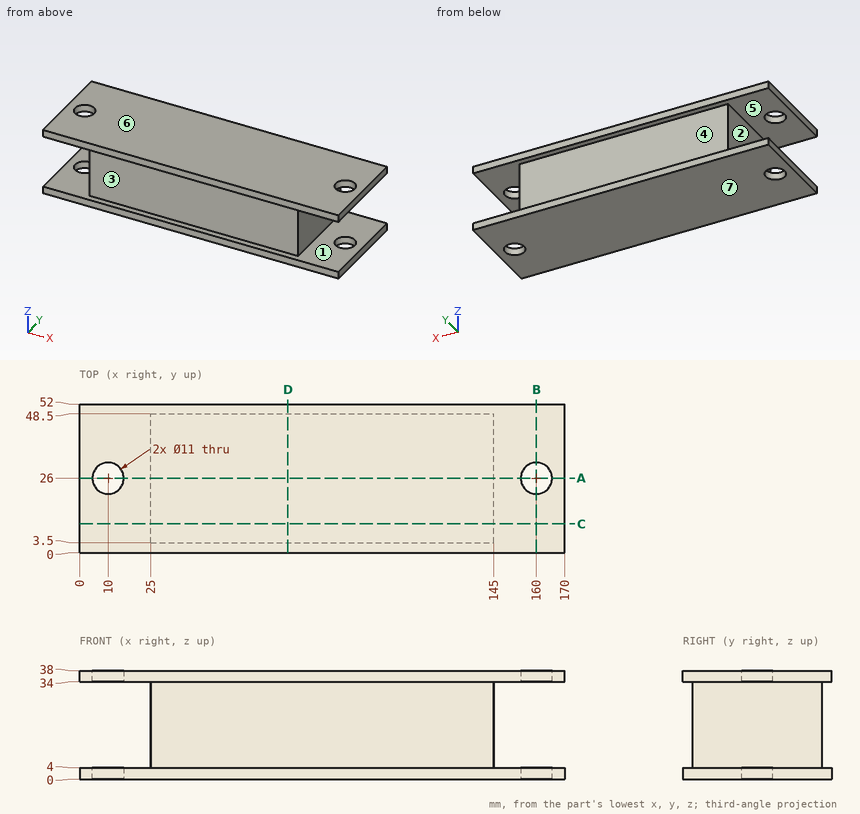
The drawing under review shows one solid part. Ordinate dimensions are in mm from its lowest x, y, z. A direction names the side the tool comes from. Coordinates: 2 decimals unless noted, no trailing zeros. Order: outer loops, then holes, each group sorted by start corner. A loop starts at its lowest first (then second) coordinate and runs counter-clockwise, first axis right, second up. Notation, with made-up numbers: (0.25, 74) -> (27.25, 74) arc R29 ccw to (27.25, 113) -> close; hole circle Ø1 at (5.5, 70.25). An arc over 180 degrees is marked (long way). Return JSON: item names as keys, results as strings.
1. For pin 1 Ø12 at (x, z) = (28, 23) entering from +Y; pin 2 Ø12 at (x, z) = (19, 33) entering from -Y; pin 3 Ø6 at (y, z) = (20, 25.5) entering from +X; pin 4 Ø8 at (x, z) = (133.5, 14.5) entering from -Y, all flat-tipped, find the tip position at first contact; note any pin that passes through.
Answer block:
{"pin 1": "y = 48.5", "pin 2": "y = 0", "pin 3": "x = 145", "pin 4": "y = 3.5"}
2. The part is to be moulded in two halves that separate along Z. For the marked faces 5, 6 and 7, say which applies: +Z half, -Z half, draft (parallel to the pull), parting line (faces both ways), or undercut.
Answer block:
{"face 5": "undercut", "face 6": "+Z half", "face 7": "-Z half"}
3. For line 1 (Y direction, x = 10, z = 35); line 2 (Z direction, x = 161, y = 17); line 3 (X direction, y = 40, z = 30.5), list the stretches that pass through material, from the lowest coordinate up. Write a range as from..to.
Answer block:
{"line 1": "0..20.5, 31.5..52", "line 2": "0..4, 34..38", "line 3": "25..145"}
4. We need section C-C on y = 10. Write out the cut boundary in (x, z), and give its area (3 significant figures).
Answer block:
{"outline": "(0, 0) -> (170, 0) -> (170, 4) -> (145, 4) -> (145, 34) -> (170, 34) -> (170, 38) -> (0, 38) -> (0, 34) -> (25, 34) -> (25, 4) -> (0, 4) -> close", "area": "4,960 mm²"}
5. Machinability: for the marked faces 1, 2, 3 and 4, which of the approach directions +Z, -Z, +X, -X, +Y, -Y give a long, thin tool a straight path to every point of the face, cutting with its end or side? Answer none if there is none.
Answer block:
{"face 1": "none", "face 2": "-X, +Y, -Y", "face 3": "+X, -X, -Y", "face 4": "+X, -X, +Y"}
6. We need section D-D on x = 73. Write out the cut boundary in (y, z).
Answer block:
{"outline": "(0, 0) -> (52, 0) -> (52, 4) -> (48.5, 4) -> (48.5, 34) -> (52, 34) -> (52, 38) -> (0, 38) -> (0, 34) -> (3.5, 34) -> (3.5, 4) -> (0, 4) -> close"}
7. We need section B-B on x = 160. Write out the cut boundary in (y, z).
Answer block:
{"outline": "(0, 0) -> (20.5, 0) -> (20.5, 4) -> (0, 4) -> close; (0, 34) -> (20.5, 34) -> (20.5, 38) -> (0, 38) -> close; (31.5, 0) -> (52, 0) -> (52, 4) -> (31.5, 4) -> close; (31.5, 34) -> (52, 34) -> (52, 38) -> (31.5, 38) -> close"}
8. We need section A-A on y = 26. Write out the cut boundary in (x, z).
Answer block:
{"outline": "(0, 0) -> (4.5, 0) -> (4.5, 4) -> (0, 4) -> close; (0, 34) -> (4.5, 34) -> (4.5, 38) -> (0, 38) -> close; (15.5, 0) -> (154.5, 0) -> (154.5, 4) -> (145, 4) -> (145, 34) -> (154.5, 34) -> (154.5, 38) -> (15.5, 38) -> (15.5, 34) -> (25, 34) -> (25, 4) -> (15.5, 4) -> close; (165.5, 0) -> (170, 0) -> (170, 4) -> (165.5, 4) -> close; (165.5, 34) -> (170, 34) -> (170, 38) -> (165.5, 38) -> close"}
